Build history of the part. All positions in model axes, mm. Face numbers are marked on the shaded views. A direction names the side the tool comes from. Round coordinates to 2 decimals unless told otherwise and drop trailing zeros. Write each loop counter-clockwise with the first axis right and the second up, starting at its lowest first coordinate (ties: lowest second). Pieces come first, ordered by that corner, then holes. Notation, with made-up numbers: (-32.75, 85) -> (18.25, 85) arc R19 cw to (18.25, 107) -> close; hole circle Ø2 at (-27, 9.5). An arc over 180 degrees is marked (long way). Return JSON: item names as keys, results as strings.
from build123d import *

# Parameters (mm, degrees)
BOSS_EXTRUDE1_DEPTH = 18
CHAMFER1_SIZE       = 3
CUT_EXTRUDE1_DEPTH  = 20
CUT_EXTRUDE3_DEPTH  = 4
SKETCH3_W           = 25
SKETCH3_H           = 6
CUT_EXTRUDE2_DEPTH  = 46.543934832
SKETCH5_W           = 28
SKETCH5_H           = 10
CUT_EXTRUDE4_DEPTH  = 46.543934832
FILLET1_R           = 3
CHAMFER2_SIZE       = 1


with BuildPart() as part:
    # Sketch1 → Boss-Extrude1 (new body)
    with BuildSketch(Plane.XY):
        Polygon((0, 17.5), (0, 0), (38, 0), (38, 4), (10, 17.5), align=None)
    extrude(amount=BOSS_EXTRUDE1_DEPTH)

    # Chamfer1
    chamfer1_edges = [part.edges().sort_by_distance(p)[0] for p in [
        (24, 10.75, 18),
    ]]
    chamfer(chamfer1_edges, length=CHAMFER1_SIZE)

    # Sketch2 → Cut-Extrude1 (cut)
    with BuildSketch(Plane(origin=(0, 17.5, 0), x_dir=(1, 0, 0), z_dir=(0, 1, 0))):
        with BuildLine():
            Line((2.75, -10), (2.75, -7))
            ThreePointArc((2.75, -7), (5, -4.75), (7.25, -7))
            Line((7.25, -7), (7.25, -10))
            ThreePointArc((7.25, -10), (5, -12.25), (2.75, -10))
        make_face()
    extrude(amount=-CUT_EXTRUDE1_DEPTH, mode=Mode.SUBTRACT)

    # Sketch4 → Cut-Extrude3 (cut)
    with BuildSketch(Plane(origin=(0, 17.5, 0), x_dir=(1, 0, 0), z_dir=(0, 1, 0))):
        with BuildLine():
            Line((9, -7), (9, -10))
            ThreePointArc((9, -10), (5, -14), (1, -10))
            Line((1, -10), (1, -7))
            ThreePointArc((1, -7), (5, -3), (9, -7))
        make_face()
    extrude(amount=-CUT_EXTRUDE3_DEPTH, mode=Mode.SUBTRACT)

    # Sketch3 → Cut-Extrude2 (cut, through all)
    with BuildSketch(Plane.XY.offset(18)):
        with Locations((12.5, 3)):
            Rectangle(SKETCH3_W, SKETCH3_H)
    extrude(amount=-CUT_EXTRUDE2_DEPTH, mode=Mode.SUBTRACT)

    # Sketch5 → Cut-Extrude4 (cut, through all)
    with BuildSketch(Plane(origin=(0, 17.5, 0), x_dir=(-1, 0, 0), z_dir=(0, 1, 0))):
        with Locations((-24, 5)):
            Rectangle(SKETCH5_W, SKETCH5_H)
    extrude(amount=-CUT_EXTRUDE4_DEPTH, mode=Mode.SUBTRACT)

    # Fillet1
    fillet1_edges = [part.edges().sort_by_distance(p)[0] for p in [
        (10, 11.75, 10),
    ]]
    fillet(fillet1_edges, radius=FILLET1_R)

    # Chamfer2
    chamfer2_edges = [part.edges().sort_by_distance(p)[0] for p in [
        (0, 11.75, 0),
        (10, 11.75, 0),
    ]]
    chamfer(chamfer2_edges, length=CHAMFER2_SIZE)


solid = part.part
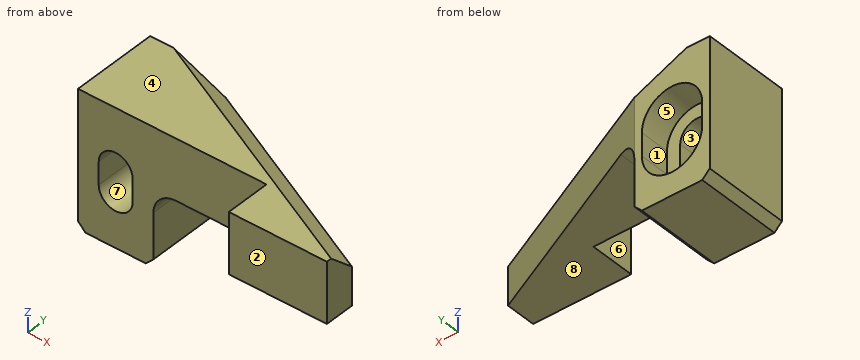
Q1. Pin check, flat tips, straight feed: pin 1 Ø3 at (x, z) = (14, 8) entering from +Y; pin 2 Ø3.5 at (y, z) = (9.5, 8) entering from +X; pin 3 Ø1 at (x, z) = (10.5, 13.5) entering from -Y; pin 4 Ø8 at (x, z) = (16, 8) entering from +Y. Stop position of each tip, or through.
Verdict:
{"pin 1": "passes through", "pin 2": "stops at x = 11.8", "pin 3": "stops at y = 6", "pin 4": "stops at y = 16.29"}
Q2. Saw through at C-C on x = 5. List the corners of the cut face in (y, z).
Verdict:
{"outline": "(6, 0) -> (17.5, 0) -> (17.5, 3) -> (13.5, 3) -> (13.5, 4.75) -> (6, 4.75) -> close; (6, 12.25) -> (13.5, 12.25) -> (13.5, 14) -> (17.5, 14) -> (17.5, 17.17) -> (16.58, 18) -> (6, 18) -> close"}
Q3. Saw through at B-B on y = 11.75. List the corners of the cut face in (x, z).
Verdict:
{"outline": "(0, 1) -> (1, 0) -> (9, 0) -> (10, 1) -> (10, 7) arc R3 cw to (13, 10) -> (21.93, 10) -> (21.93, 15) -> (15.02, 18) -> (0, 18) -> close; hole (2.75, 7) arc R2.25 ccw to (7.25, 7) -> (7.25, 10) arc R2.25 ccw to (2.75, 10) -> close"}
Q4. Wall check: L1, parallel to Z at x = 27.5, y = 2; L2, parallel to X at y = 3.75, z = 11.5; L3, parallel to Y at x = 7.5, z = 2.5. Give the ranges that are in metal, low to high.
Verdict:
{"L1": "z = 10 to 18", "L2": "x = 25 to 38", "L3": "y = 6 to 17.5"}
Q5. Saw through at D-D on z = 17.25. List the corners of the cut face in (x, y), then the cut area to 3 significant figures.
Verdict:
{"outline": "(0, 6) -> (25, 6) -> (25, 0) -> (38, 0) -> (38, 1.5) -> (4.82, 17.5) -> (0, 17.5) -> close", "area": "250 mm²"}
Q6. 3-axis set-ups, long thin cutter, end or side, ignore diameter. For the marked faces 5, 6, 7 and 8: which of +Z, -Z, +X, -X, +Y, -Y reach the whole face in a straight line?
Verdict:
{"face 5": "+Y", "face 6": "+Z, -Z, -X, -Y", "face 7": "+Y, -Y", "face 8": "-Z, +X, +Y, -Y"}
Q7. Two-plate mould, pull along Z, no slides. Class the marked faces 1, 2, 3 and 4: +Z half, -Z half, draft (parallel to the pull), parting line (faces both ways), or undercut.
Verdict:
{"face 1": "undercut", "face 2": "draft", "face 3": "undercut", "face 4": "+Z half"}
Q8. Saw through at A-A on z = 11. List the corners of the cut face in (x, y), then the cut area to 3 significant figures.
Verdict:
{"outline": "(0, 6) -> (2.98, 6) -> (2.98, 13.5) -> (1.13, 13.5) -> (1.13, 17.5) -> (0, 17.5) -> close; (7.02, 6) -> (25, 6) -> (25, 0) -> (38, 0) -> (38, 4) -> (10, 17.5) -> (8.87, 17.5) -> (8.87, 13.5) -> (7.02, 13.5) -> close", "area": "265 mm²"}
